from build123d import *

# Parameters (mm, degrees)
SKETCH_13_W               = 12
SKETCH_13_H               = 70
EXTRUDE_1_DEPTH           = 45
HOLE_WIZARD_M3_1_D        = 2.5
HOLE_WIZARD_M3_1_DEPTH    = 12.5
HOLE_WIZARD_M3_1_TIP      = 0.751075774
HOLE_WIZARD_M5_1_D        = 4.2
HOLE_WIZARD_M5_1_DEPTH    = 19
HOLE_WIZARD_M5_1_TIP      = 1.2618073
HOLE_WIZARD_1_D           = 6.4
HOLE_WIZARD_1_CBORE_D     = 11
HOLE_WIZARD_1_CBORE_DEPTH = 20
HOLE_WIZARD_6_0_6_1_D     = 6
HOLE_WIZARD_6_0_6_1_DEPTH = 10
HOLE_WIZARD_6_0_6_1_TIP   = 1.802581857
HOLE_WIZARD_6_0_6_2_D     = 6
HOLE_WIZARD_6_0_6_2_DEPTH = 10
HOLE_WIZARD_6_0_6_2_TIP   = 1.802581857


with BuildPart() as part:
    # 草图13 → 凸台-拉伸1 (new body)
    with BuildSketch(Plane.XY):
        Rectangle(SKETCH_13_W, SKETCH_13_H)
    extrude(amount=EXTRUDE_1_DEPTH)

    # M3 螺纹孔1
    with Locations(Plane(origin=(0, 35, 0), x_dir=(1, 0, 0), z_dir=(0, 1, 0))):
        with Locations((0, -10), (0, -16)):
            Hole(HOLE_WIZARD_M3_1_D / 2, depth=HOLE_WIZARD_M3_1_DEPTH)
            with Locations((0, 0, -(HOLE_WIZARD_M3_1_DEPTH + HOLE_WIZARD_M3_1_TIP / 2))):  # 118° drill point
                Cone(0, HOLE_WIZARD_M3_1_D / 2, HOLE_WIZARD_M3_1_TIP, mode=Mode.SUBTRACT)

    # M5 螺纹孔1
    with Locations(Plane.XY.offset(45)):
        with Locations((0, 31), (0, -31)):
            Hole(HOLE_WIZARD_M5_1_D / 2, depth=HOLE_WIZARD_M5_1_DEPTH)
            with Locations((0, 0, -(HOLE_WIZARD_M5_1_DEPTH + HOLE_WIZARD_M5_1_TIP / 2))):  # 118° drill point
                Cone(0, HOLE_WIZARD_M5_1_D / 2, HOLE_WIZARD_M5_1_TIP, mode=Mode.SUBTRACT)

    # 打孔尺寸(%根据)内六角圆柱头螺钉的类型1 (through all)
    with Locations(Plane.XY.offset(45)):
        with Locations((0, 13), (0, -13)):
            CounterBoreHole(HOLE_WIZARD_1_D / 2, HOLE_WIZARD_1_CBORE_D / 2, HOLE_WIZARD_1_CBORE_DEPTH)

    # Ø6.0 (6) 直径孔1
    with Locations(Plane.XY.offset(45)):
        with Locations((0, 0)):
            Hole(HOLE_WIZARD_6_0_6_1_D / 2, depth=HOLE_WIZARD_6_0_6_1_DEPTH)
            with Locations((0, 0, -(HOLE_WIZARD_6_0_6_1_DEPTH + HOLE_WIZARD_6_0_6_1_TIP / 2))):  # 118° drill point
                Cone(0, HOLE_WIZARD_6_0_6_1_D / 2, HOLE_WIZARD_6_0_6_1_TIP, mode=Mode.SUBTRACT)

    # Ø6.0 (6) 直径孔2
    with Locations(Plane(origin=(0, 0, 0), x_dir=(-1, 0, 0), z_dir=(0, 0, -1))):
        with Locations((0, -22.5), (0, 22.5)):
            Hole(HOLE_WIZARD_6_0_6_2_D / 2, depth=HOLE_WIZARD_6_0_6_2_DEPTH)
            with Locations((0, 0, -(HOLE_WIZARD_6_0_6_2_DEPTH + HOLE_WIZARD_6_0_6_2_TIP / 2))):  # 118° drill point
                Cone(0, HOLE_WIZARD_6_0_6_2_D / 2, HOLE_WIZARD_6_0_6_2_TIP, mode=Mode.SUBTRACT)


solid = part.part
For this review, take the finished solid that the model builds, in its own axes (mm). A direction names the side the tool comes from. Coordinates: 2 decimals unless noted, no trailing zeros. Loops run counter-clockwise (first coordinate to the right, second up) from the corner with the lowest first, then second, coordinate; pieces in that order, holes last. Notation, with made-up numbers: (57, 67.5) - (84, 67.5) arc R23 cw to (84, 97.5) - close; hole circle Ø2 at (-32.5, 64.5). An arc over 180 degrees is marked (long way). Use a Markdown table: item, result. Add a question column.
Item 1: Insertion check: pin 1 Ø2 at (x, y) = (3, -3) entering from -Z; pin 2 Ø3.5 at (x, y) = (0, -22.5) entering from -Z; pin 3 Ø6.5 at (x, y) = (0, -13) entering from +Z; pin 4 Ø2 at (x, z) = (0, 16) entering from +Y. Each pin has a flat end and moves straight along its axis. Give the tip position at first contact, or say it passes through.
Item 2: Tool access review of faces 5 (the face through (-0.65, 19.57, 5.07)), 6 (the face through (3, 0, 40)), 7 (the face through (0.694, -16.124, 12.325)): name each direction out of +Z, -Z, +X, -X, +Y, -Y from which nothing blocks a thin tool from reaching the whole face with its end or side.
Item 3: Mouldability with a two-part tool opening along Y and no side actions: class faces 1 (the face through (-0.047, -30.638, 24.957)), 2 (the face through (0, 35, 22)), 3 (the face through (0.11, 21.99, 11.49)), 4 (the face through (0.27, 29.13, 11.22)) as pulls with the +Y half, pulls with the -Y half, needs draft (parallel to the pull), parting line crosses it, or undercut.
Item 4: For line 1 (Y direction, x = 0, z = 39.5); line 2 (Y direction, x = 0, z = 5); line 3 (X direction, y = 30, z = 10), list the stretches that pass through material, from the lowest coordinate up.
Item 5: We need section C-C (z = 19). Give the boundary of the cut face in (x, y), and give its area (3 significant figures).
Item 6: We need section B-B (y = -13). Give the boundary of the cut face in (x, z).
Item 7: We need section A-A (z = 36). Give the boundary of the cut face in (x, y), and give its area (3 significant figures).
Item 8: We need section D-D (z = 27.5). Give the boundary of the cut face in (x, y), and give its area (3 significant figures).
Results list:
| question | item | result |
|---|---|---|
| 1 | pin 1 | stops at z = 0 |
| 1 | pin 2 | stops at z = 10.75 |
| 1 | pin 3 | stops at z = 25 |
| 1 | pin 4 | stops at y = 22.35 |
| 2 | face 5 | -Z |
| 2 | face 6 | +Z |
| 2 | face 7 | +Z, -Z |
| 3 | face 1 | undercut |
| 3 | face 2 | pulls with the +Y half |
| 3 | face 3 | undercut |
| 3 | face 4 | needs draft |
| 4 | line 1 | y = -35 to -33.1, -28.9 to -18.5, -7.5 to -3, 3 to 7.5, 18.5 to 28.9, 33.1 to 35 |
| 4 | line 2 | y = -35 to -25.5, -19.5 to -16.2, -9.8 to 9.8, 16.2 to 19.5, 25.5 to 35 |
| 4 | line 3 | x = -6 to -1.25, 1.25 to 6 |
| 5 | outline | (-6, -35) - (6, -35) - (6, 35) - (-6, 35) - close; hole circle Ø6.4 at (0, -13); hole circle Ø6.4 at (0, 13) |
| 5 | area | 776 mm^2 |
| 6 | outline | (-6, 0) - (-3.2, 0) - (-3.2, 25) - (-5.5, 25) - (-5.5, 45) - (-6, 45) - close; (3.2, 0) - (6, 0) - (6, 45) - (5.5, 45) - (5.5, 25) - (3.2, 25) - close |
| 7 | outline | (-6, -35) - (6, -35) - (6, 35) - (-6, 35) - close; hole circle Ø11 at (0, -13); hole circle Ø11 at (0, 13); hole circle Ø6 at (0, 0); hole circle Ø4.2 at (0, -31); hole circle Ø4.2 at (0, 31) |
| 7 | area | 594 mm^2 |
| 8 | outline | (-6, -35) - (6, -35) - (6, 35) - (-6, 35) - close; hole circle Ø11 at (0, -13); hole circle Ø11 at (0, 13); hole circle Ø4.2 at (0, -31); hole circle Ø4.2 at (0, 31) |
| 8 | area | 622 mm^2 |
